Verification items for the finished model (mm, model axes). A direction names the side the tool comes from. Round coordinates to 2 decimals unless told otherwise and drop trailing zeros. Order: outer loops, then holes, each group sorted by start corner. A loop starts at its lowest first (then second) coordinate and runs counter-clockwise, first axis right, second up. Notation, with made-up numbers: M 6.5,72.25 L 57.5,72.25 A10 cw 57.5,77.25 Z; hole C 5.5,24 d1. An arc over 180 degrees is marked long. Return JSON: item names as keys, results as strings. Group by question number.
from build123d import *

# Parameters (mm, degrees)
SKETCH1_R                   = 2.5
SKETCH1_R_2                 = 2
SKETCH1_W                   = 50
SKETCH1_H                   = 20
BOSS_EXTRUDE1_DEPTH         = 8
CHAMFER1_SIZE               = 3
TAP_DRILL_FOR_M8_TAP1_D     = 6.8
TAP_DRILL_FOR_M8_TAP1_DEPTH = 15
TAP_DRILL_FOR_M8_TAP1_TIP   = 2.042926105
TAP_DRILL_FOR_M5_TAP1_D     = 4.2
TAP_DRILL_FOR_M5_TAP1_DEPTH = 15
TAP_DRILL_FOR_M5_TAP1_TIP   = 1.2618073
CUT_EXTRUDE1_DEPTH          = 10
LPATTERN1_COUNT             = 2
LPATTERN1_PITCH             = 20


with BuildPart() as part:
    # Sketch1 → Boss-Extrude1 (new body)
    with BuildSketch(Plane.XY):
        Polygon((0, 180), (10, 190), (90, 190), (100, 180), (100, 10), (90, 0), (10, 0), (0, 10), align=None)
        with Locations((35, 6)):
            Circle(SKETCH1_R, mode=Mode.SUBTRACT)
        with Locations((65, 6)):
            Circle(SKETCH1_R, mode=Mode.SUBTRACT)
        with Locations((22.5, 125)):
            Circle(SKETCH1_R_2, mode=Mode.SUBTRACT)
        with Locations((50, 125)):
            Circle(SKETCH1_R_2, mode=Mode.SUBTRACT)
        with Locations((77.5, 125)):
            Circle(SKETCH1_R_2, mode=Mode.SUBTRACT)
        with Locations((50, 25)):
            Rectangle(SKETCH1_W, SKETCH1_H, mode=Mode.SUBTRACT)
        with BuildLine():
            Line((56, 70), (56, 50))
            ThreePointArc((56, 50), (50, 44), (44, 50))
            Line((44, 50), (44, 70))
            ThreePointArc((44, 70), (50, 76), (56, 70))
        make_face(mode=Mode.SUBTRACT)
    extrude(amount=BOSS_EXTRUDE1_DEPTH)

    # Chamfer1
    chamfer1_edges = [part.edges().sort_by_distance(p)[0] for p in [
        (25, 35, 4),
        (25, 15, 4),
        (75, 15, 4),
        (75, 35, 4),
    ]]
    chamfer(chamfer1_edges, length=CHAMFER1_SIZE)

    # Tap Drill for M8 Tap1
    with Locations(Plane(origin=(25, 60, 8), x_dir=(1, 0, 0), z_dir=(0, 0, 1))):
        with Locations((0, 0), (50, 0)):
            Hole(TAP_DRILL_FOR_M8_TAP1_D / 2, depth=TAP_DRILL_FOR_M8_TAP1_DEPTH)
            with Locations((0, 0, -(TAP_DRILL_FOR_M8_TAP1_DEPTH + TAP_DRILL_FOR_M8_TAP1_TIP / 2))):  # 118° drill point
                Cone(0, TAP_DRILL_FOR_M8_TAP1_D / 2, TAP_DRILL_FOR_M8_TAP1_TIP, mode=Mode.SUBTRACT)

    # Tap Drill for M5 Tap1
    with Locations(Plane(origin=(94, 23.685438565, 0), x_dir=(-1, 0, 0), z_dir=(0, 0, -1))):
        with Locations((0, 0), (88, 0)):
            Hole(TAP_DRILL_FOR_M5_TAP1_D / 2, depth=TAP_DRILL_FOR_M5_TAP1_DEPTH)
            with Locations((0, 0, -(TAP_DRILL_FOR_M5_TAP1_DEPTH + TAP_DRILL_FOR_M5_TAP1_TIP / 2))):  # 118° drill point
                Cone(0, TAP_DRILL_FOR_M5_TAP1_D / 2, TAP_DRILL_FOR_M5_TAP1_TIP, mode=Mode.SUBTRACT)

    # Sketch5 → Cut-Extrude1 (cut)
    with BuildSketch(Plane(origin=(0, 0, 0), x_dir=(-1, 0, 0), z_dir=(0, 0, -1))):
        with BuildLine():
            Line((-85, 178.5), (-65, 178.5))
            ThreePointArc((-65, 178.5), (-61.5, 175), (-65, 171.5))
            Line((-65, 171.5), (-85, 171.5))
            ThreePointArc((-85, 171.5), (-88.5, 175), (-85, 178.5))
        make_face()
        with BuildLine():
            Line((-15, 178.5), (-35, 178.5))
            ThreePointArc((-35, 178.5), (-38.5, 175), (-35, 171.5))
            Line((-35, 171.5), (-15, 171.5))
            ThreePointArc((-15, 171.5), (-11.5, 175), (-15, 178.5))
        make_face()
    cut_extrude1 = extrude(amount=-CUT_EXTRUDE1_DEPTH, mode=Mode.SUBTRACT)

    # LPattern1: Cut-Extrude1 ×2
    with Locations(*[(0, -i * LPATTERN1_PITCH, 0) for i in range(1, LPATTERN1_COUNT)]):
        add(cut_extrude1, mode=Mode.SUBTRACT)


solid = part.part
1. Cross-section at A-A (y = 60). Enter the section's corners in (x, z).
2. Draft check along Y on faces 1 (the face through (100, 96, 4)), 2 (the face through (91.902, 23.778, 4.056)), 3 (the face through (5, 5, 4)), 4 (the face through (50, 15, 4)). Enter one of: +Y half, -Y half, draft (parallel to the pull), parting line (faces both ways), or undercut.
3. Cross-section at D-D (z = 1.75). Give the number of separate pieces and of enclosed holes in the cut face, plus the area to 3 significant figures.
4. Thickness scan on line 1 along Y through (x, z) = (65, 4.25); line 2 along Y through (x, z) = (70, 4); line 3 along X through (y, z) = (23.5, 3.5). Record the ranges inside material, lowest first. Write a range as from..to.
5. Access from +Z, -Z, +X, -X, +Y, -Y to the whole of each face (thin tool, end or side, straight path). Record for faces 5 (the face through (25, 25, 4)), 6 (the face through (51, 96, 8)).
6. Cross-section at B-B (y = 155). Enter the section's corners in (x, z).
7. Cross-section at C-C (x = 6). Enter the section's corners in (y, z).
8. Go/stop test with a flat-tipped pin: pin 1 (6.5 mm diameter, centred on x = 65, y = 6, fed in from +Z). Record where the tip stops, or that it passes through.
Computed:
{
 "1": {"outline": "M 0,0 L 21.6,0 L 21.6,8 L 0,8 Z; M 28.4,0 L 44,0 L 44,8 L 28.4,8 Z; M 56,0 L 71.6,0 L 71.6,8 L 56,8 Z; M 78.4,0 L 100,0 L 100,8 L 78.4,8 Z"},
 "2": {"face 1": "draft", "face 2": "undercut", "face 3": "-Y half", "face 4": "undercut"},
 "3": {"separate pieces": "1", "enclosed holes": "15", "area": "16,600 mm²"},
 "4": {"line 1": "y = 0..3.5, 8.5..15, 35..151.5, 158.5..171.5, 178.5..190", "line 2": "y = 0..15, 35..151.5, 158.5..171.5, 178.5..190", "line 3": "x = 0..3.91, 8.09..25, 75..91.91, 96.09..100"},
 "5": {"face 5": "+Z, -Z", "face 6": "+Z, +X, -X, +Y, -Y"},
 "6": {"outline": "M 0,0 L 11.5,0 L 11.5,8 L 0,8 Z; M 38.5,0 L 61.5,0 L 61.5,8 L 38.5,8 Z; M 88.5,0 L 100,0 L 100,8 L 88.5,8 Z"},
 "7": {"outline": "M 4,0 L 21.59,0 L 21.59,8 L 4,8 Z; M 25.79,0 L 186,0 L 186,8 L 25.79,8 Z"},
 "8": {"pin 1": "stops at z = 8"}
}
